Can you work these out from the model? Positions are in its coordinate system, mm. Face numbers are marked on the shaded views. A direction names the side the tool comes from. Give positions to 0.01 mm unless a question says otherwise; leave off trailing zeros. Loops run counter-clockwise (first coordinate to the right, second up) from the corner with the lowest first, then second, coordinate; pieces in that order, holes last.
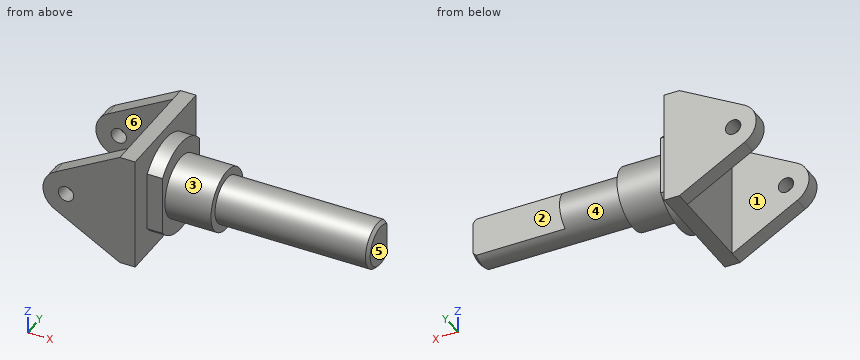
from build123d import *

# Parameters (mm, degrees)
BASE_PLATE_SKETCH_W         = 10
BASE_PLATE_SKETCH_H         = 76
BASE_PLATE_DEPTH            = 74
FORK_EAR_1_DEPTH            = 10
FORK_START                  = -10
FORK_EAR_2_DEPTH            = 10
PIVOT_PIN_HOLE_SKETCH_R     = 5
PIVOT_PIN_HOLE_10_DEPTH     = 100
HEX_COLLAR_DEPTH            = 10
SHOULDER_40_SKETCH_R        = 20
SHOULDER_40_DEPTH           = 30
SHAFT_30_SKETCH_R           = 15
SHAFT_30_DEPTH              = 100
SHAFT_START                 = -60
SHAFT_FLAT_DEPTH            = 60
SHAFT_END_CHAMFER_2X45_SIZE = 2


with BuildPart() as part:
    # Base Plate Sketch → Base Plate (new body)
    with BuildSketch(Plane.XY):
        with Locations((-5, 0)):
            Rectangle(BASE_PLATE_SKETCH_W, BASE_PLATE_SKETCH_H)
    extrude(amount=-BASE_PLATE_DEPTH)

    # Fork Ear 1 Sketch → Fork Ear 1 (add)
    with BuildSketch(Plane(origin=(0, 38, 0), x_dir=(1, 0, 0), z_dir=(0, 1, 0))):
        with BuildLine():
            Line((-10, 74), (-10, 0))
            Line((-10, 0), (-52.377859531, 23.939862606))
            ThreePointArc((-52.377859531, 23.939862606), (-60, 37), (-52.377859531, 50.060137394))
            Line((-52.377859531, 50.060137394), (-10, 74))
        make_face()
    extrude(amount=-FORK_EAR_1_DEPTH)

    # Fork Ear 2 Sketch → Fork Ear 2 (add)
    with BuildSketch(Plane.XZ.offset(38).offset(FORK_START)):
        with BuildLine():
            Line((-52.377859531, -23.939862606), (-10, 0))
            Line((-10, 0), (-10, -74))
            Line((-10, -74), (-52.377859531, -50.060137394))
            ThreePointArc((-52.377859531, -50.060137394), (-60, -37), (-52.377859531, -23.939862606))
        make_face()
    extrude(amount=FORK_EAR_2_DEPTH)

    # Pivot Pin Hole Sketch → Pivot Pin Hole Ø10 (cut)
    with BuildSketch(Plane.XZ.offset(38)):
        with Locations(Location((-45, -37, 0), (0, 0, 270))):
            Circle(PIVOT_PIN_HOLE_SKETCH_R)
    extrude(amount=-PIVOT_PIN_HOLE_10_DEPTH, mode=Mode.SUBTRACT)

    # Hex Collar Sketch → Hex Collar (add)
    with BuildSketch(Plane(origin=(0, 0, 0), x_dir=(0, 0, -1), z_dir=(1, 0, 0))):
        with BuildLine():
            Line((17.738639716, 23), (56.261360284, 23))
            ThreePointArc((56.261360284, 23), (67, 0), (56.261360284, -23))
            Line((56.261360284, -23), (17.738639716, -23))
            ThreePointArc((17.738639716, -23), (7, 0), (17.738639716, 23))
        make_face()
    extrude(amount=HEX_COLLAR_DEPTH)

    # Shoulder Ø40 Sketch → Shoulder Ø40 (add)
    with BuildSketch(Plane(origin=(10, 0, 0), x_dir=(0, 0, -1), z_dir=(1, 0, 0))):
        with Locations((37, 0)):
            Circle(SHOULDER_40_SKETCH_R)
    extrude(amount=SHOULDER_40_DEPTH)

    # Shaft Ø30 Sketch → Shaft Ø30 (add)
    with BuildSketch(Plane(origin=(40, 0, 0), x_dir=(0, 0, -1), z_dir=(1, 0, 0))):
        with Locations((37, 0)):
            Circle(SHAFT_30_SKETCH_R)
    extrude(amount=SHAFT_30_DEPTH)

    # Shaft Flat Sketch → Shaft Flat (cut)
    with BuildSketch(Plane(origin=(140, 0, 0), x_dir=(0, 0, -1), z_dir=(1, 0, 0)).offset(SHAFT_START)):
        with BuildLine():
            Line((24.31142246, 8), (49.68857754, 8))
            ThreePointArc((49.68857754, 8), (37, 15), (24.31142246, 8))
        make_face()
    extrude(amount=SHAFT_FLAT_DEPTH, mode=Mode.SUBTRACT)

    # Shaft End Chamfer 2x45°
    shaft_end_chamfer_2x45_edges = [part.edges().sort_by_distance(p)[0] for p in [
        (140, -14.410563193, -32.836387572),
    ]]
    chamfer(shaft_end_chamfer_2x45_edges, length=SHAFT_END_CHAMFER_2X45_SIZE)


solid = part.part
(1) Will these pins go through, and if not, where does the flat tip stop? P1, Ø25, axis at x = -44.5, z = -39.5, coming from the -Y side; P2, Ø4, axis at y = 18, z = -27.5, coming from the -X side; P3, Ø11, axis at x = 7, z = -45, coming from the +Y side; P4, Ø5, axis at x = 5.5, z = -30.5, coming from the -Y side.
Returned:
P1: stops at y = -38
P2: stops at x = -10
P3: stops at y = 23
P4: stops at y = -23
(2) Suppose I cut it at D-D on z = -60. List the corners of the cut face in (x, y) for me, plus the area to 3 significant figures.
Returned:
outline: (-34.78, -38) - (0, -38) - (0, -19.26) - (10, -19.26) - (10, 19.26) - (0, 19.26) - (0, 38) - (-34.78, 38) - (-34.78, 28) - (-10, 28) - (-10, -28) - (-34.78, -28) - close
area: 1,640 mm2
(3) Which directions (+Z, -Z, +X, -X, +Y, -Y) give clear straight access to the entire face, cutting with the end or side of a thin tool? Please do the marked faces 1, 2 and 3.
Returned:
face 1: +Z, -Z, -X
face 2: +Z, -Z, +X, +Y
face 3: +X
(4) Suppose I cut it at C-C on x = -45. List the corners of the cut face in (y, z) for me, plus the area to 3 significant figures.
Returned:
outline: (-38, -54.23) - (-28, -54.23) - (-28, -42) - (-38, -42) - close; (-38, -32) - (-28, -32) - (-28, -19.77) - (-38, -19.77) - close; (28, -54.23) - (38, -54.23) - (38, -42) - (28, -42) - close; (28, -32) - (38, -32) - (38, -19.77) - (28, -19.77) - close
area: 489 mm2
(5) Thinking about a two-plate mould opening in Y: for the marked faces 4, 5 and 6, which applies, pulls with the +Y half, pulls with the -Y half, needs draft (parallel to the pull), parting line crosses it, or undercut?
Returned:
face 4: parting line crosses it
face 5: needs draft
face 6: undercut
(6) Suppose I cut it at B-B on y = 0. List the corners of the cut face in (x, z) for me, plus the area to 3 significant figures.
Returned:
outline: (-10, -74) - (0, -74) - (0, -67) - (10, -67) - (10, -57) - (40, -57) - (40, -52) - (138, -52) - (140, -50) - (140, -24) - (138, -22) - (40, -22) - (40, -17) - (10, -17) - (10, -7) - (0, -7) - (0, 0) - (-10, 0) - close
area: 5,540 mm2
(7) Suppose I cut it at A-A on z = -37. Give the number of separate pieces and of enclosed holes in the cut face, plus the area to 3 significant figures.
Returned:
separate pieces: 3
enclosed holes: 0
area: 5,800 mm2
(8) Please list where these lines run through material, in increasing order: probe 1 along X at (y, z) = (35.5, -37); probe 2 along Y at (x, z) = (5, -55.5); probe 3 along X at (y, z) = (28.5, -46).
Returned:
probe 1: x = -60 to -50, -40 to 0
probe 2: y = -23 to 23
probe 3: x = -57 to 0
